Geometry check sheet. Reference: drawing and pictorial views, mm from the part's lowest x, y, z. A direction names the side the tool comes from. Give positions to 0.01 mm unless a question says otherwise; leave off trailing zeros. Order: outer loops, then holes, each group sorted by start corner. A loop starts at its lowest first (then second) coordinate and runs counter-clockwise, first axis right, second up. Notation, with made-up numbers: (65, 64) - (85, 64) arc R30 cw to (85, 87) - close; hole circle Ø3 at (81.5, 1). An arc over 180 degrees is marked (long way). Answer as a JSON object with one key per item and string values.
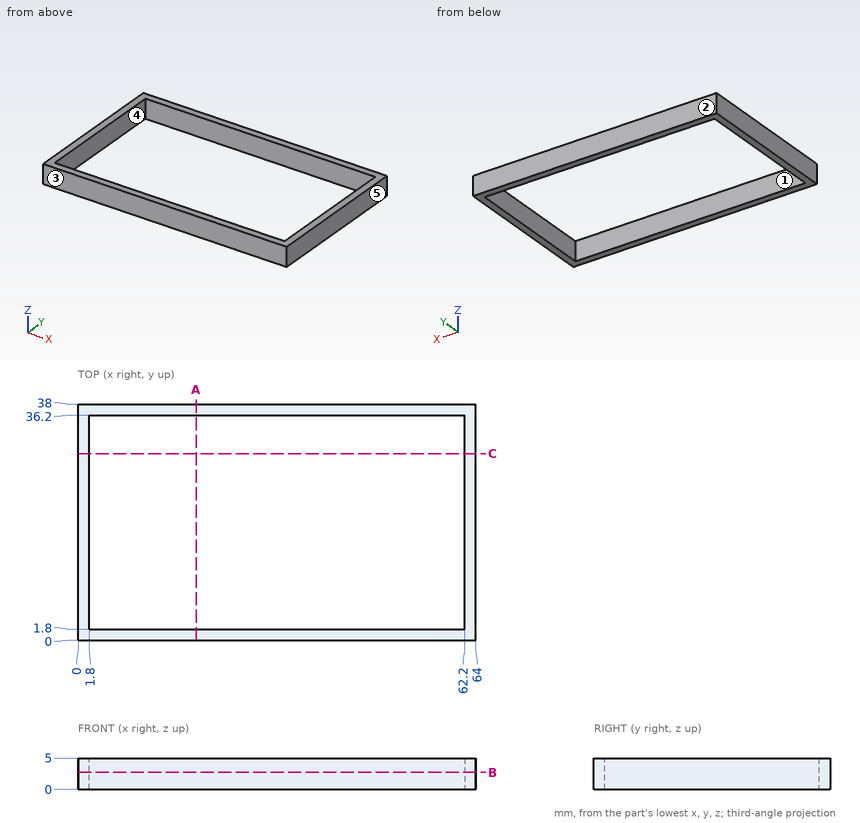
(1) Section check B-B (z = 2.7). Record the cut outline in (x, y), then the cut area to 3 significant figures.
Computed values:
{"outline": "(0, 0) - (64, 0) - (64, 38) - (0, 38) - close; hole (1.8, 1.8) - (62.2, 1.8) - (62.2, 36.2) - (1.8, 36.2) - close", "area": "354 mm²"}
(2) Release check for a two-part mould opening along Y. For the marked faces 3, 4 and 5 record: pulls with the +Y half, pulls with the -Y half, needs draft (parallel to the pull), parting line crosses it, or undercut.
Computed values:
{"face 3": "pulls with the -Y half", "face 4": "undercut", "face 5": "needs draft"}
(3) Material ranges on line 1 along X through (y, z) = (21, 1.6); line 2 along Y through (x, z) = (42, 0.8), recorded low to high. Write a range as [from, to].
Computed values:
{"line 1": "x = [0, 1.8], [62.2, 64]", "line 2": "y = [0, 1.8], [36.2, 38]"}
(4) Access from +Z, -Z, +X, -X, +Y, -Y to the whole of each face (thin tool, end or side, straight path). Record for the marked faces 1 and 2.
Computed values:
{"face 1": "+Z, -Z", "face 2": "+Z, -Z, +X, -X, +Y"}
(5) Section check C-C (y = 30). Record the cut outline in (x, z), then the cut area to 3 significant figures.
Computed values:
{"outline": "(0, 0) - (1.8, 0) - (1.8, 5) - (0, 5) - close; (62.2, 0) - (64, 0) - (64, 5) - (62.2, 5) - close", "area": "18.0 mm²"}
(6) Section check A-A (x = 19). Record the cut outline in (y, z).
Computed values:
{"outline": "(0, 0) - (1.8, 0) - (1.8, 5) - (0, 5) - close; (36.2, 0) - (38, 0) - (38, 5) - (36.2, 5) - close"}
